from build123d import *

# Parameters (mm, degrees)
BASE_PLATE_SKETCH_W          = 140
BASE_PLATE_SKETCH_H          = 85
BASE_PLATE_DEPTH             = 18
UNDERSIDE_GROOVE_SKETCH_W    = 49
UNDERSIDE_GROOVE_SKETCH_H    = 3
UNDERSIDE_GROOVE_DEPTH       = 148.411838059
BASE_HOLES_SKETCH_R          = 8
BASE_HOLES_DEPTH             = 84.846586096
UPRIGHT_LUG_PLATE_DEPTH      = 12
UPRIGHT_LUG_PLATE_DEPTH_BACK = 24
UPRIGHT_LUG_PLATE_SKETCH_R   = 27.5
UPRIGHT_LUG_PLATE_SKETCH_R_2 = 15
SIDE_GUSSET_SKETCH_R         = 20
SIDE_GUSSET_SKETCH_R_2       = 9
SIDE_GUSSET_DEPTH            = 24
HINGE_BOSS_EXTENSION_DEPTH   = 12


with BuildPart() as part:
    # Base Plate Sketch → Base Plate (new body)
    with BuildSketch(Plane(origin=(0, 0, 0), x_dir=(1, 0, 0), z_dir=(0, 1, 0))):
        Rectangle(BASE_PLATE_SKETCH_W, BASE_PLATE_SKETCH_H)
    extrude(amount=BASE_PLATE_DEPTH)

    # Underside Groove Sketch → Underside Groove (cut, through all)
    with BuildSketch(Plane(origin=(70, 0, 0), x_dir=(0, 0, -1), z_dir=(1, 0, 0))):
        with Locations((0, 1.5)):
            Rectangle(UNDERSIDE_GROOVE_SKETCH_W, UNDERSIDE_GROOVE_SKETCH_H)
    extrude(amount=-UNDERSIDE_GROOVE_DEPTH, mode=Mode.SUBTRACT)

    # Base Holes Sketch → Base Holes (cut, through all)
    with BuildSketch(Plane(origin=(0, 18, 0), x_dir=(1, 0, 0), z_dir=(0, 1, 0))):
        with Locations(Location((-35, -12.5, 0), (0, 0, 270))):
            Circle(BASE_HOLES_SKETCH_R)
        with Locations(Location((35, -12.5, 0), (0, 0, 270))):
            Circle(BASE_HOLES_SKETCH_R)
    extrude(amount=-BASE_HOLES_DEPTH, mode=Mode.SUBTRACT)



with BuildPart() as body_2:
    # Upright Lug Plate Sketch → Upright Lug Plate (new, two sides: drawn at the far end of the back side and taken through both)
    with BuildSketch(Plane(origin=(0, 0, -42.5), x_dir=(-1, 0, 0), z_dir=(0, 0, -1)).offset(-UPRIGHT_LUG_PLATE_DEPTH_BACK)):
        with Locations((-20, 118)):
            Circle(UPRIGHT_LUG_PLATE_SKETCH_R)
        with Locations((-20, 118)):
            Circle(UPRIGHT_LUG_PLATE_SKETCH_R_2, mode=Mode.SUBTRACT)
    extrude(amount=UPRIGHT_LUG_PLATE_DEPTH + UPRIGHT_LUG_PLATE_DEPTH_BACK)


with BuildPart() as body_3:
    # Side Gusset Sketch → Side Gusset (new body)
    with BuildSketch(Plane(origin=(0, 0, -42.5), x_dir=(-1, 0, 0), z_dir=(0, 0, -1))):
        with Locations((50, 56)):
            Circle(SIDE_GUSSET_SKETCH_R)
        with Locations((50, 56)):
            Circle(SIDE_GUSSET_SKETCH_R_2, mode=Mode.SUBTRACT)
    extrude(amount=-SIDE_GUSSET_DEPTH)


with BuildPart() as part_1:
    add(part.part)

    add(body_2.part)  # Hinge Boss Extension merges body 2

    add(body_3.part)  # Hinge Boss Extension merges body 3
    # Hinge Boss Extension Sketch → Hinge Boss Extension (add)
    with BuildSketch(Plane(origin=(0, 0, -42.5), x_dir=(-1, 0, 0), z_dir=(0, 0, -1))):
        with BuildLine():
            Line((70, 18), (70, 56))
            ThreePointArc((70, 56), (40.100426872, 38.621897345), (39.800154813, 73.203579806))
            ThreePointArc((39.800154813, 73.203579806), (10.05246179, 76.375791932), (4.645420553, 105.799457153))
            ThreePointArc((4.645420553, 105.799457153), (-29.103509689, 92.050508457), (-46.866088482, 123.870544241))
            Line((-46.866088482, 123.870544241), (-70, 18))
            Line((-70, 18), (70, 18))
        make_face()
    extrude(amount=-HINGE_BOSS_EXTENSION_DEPTH)


solid = part_1.part
Input: part model. Units: mm. Frame: model coordinates. A direction names the side the tool comes from. Coordinates: 2 decimals unless noted, no trailing zeros. Write each loop counter-clockwise with the first axis right and the second up, starting at its lowest first coordinate (ties: lowest second). Pieces come first, ordered by that corner, then holes. Notation, with made-up numbers: M 29,-7 L 67,-7 A17 cw 67,6 Z; hole C 58,13 d10. An arc over 180 degrees is marked long. Answer as a JSON object with one key per item and string values. Group by question number.
(1) Section A-A on z = -28. Output: boundary loops of the cut face in (x, y), plus the area to 3 significant figures.
(2) Set-up query: faces 4 (the face through (-60.752, 72.864, -28.001)), 5 (the face through (-54, 47, -18.5)), 6 (the face through (-1, 0, 33)). Return all of +Z, -Z, +X, -X, +Y, -Y with unobstructed straight access to the full face (end or side cutting, diameter ignored); none if empty.
(3) Mould query, pull axis X, two halves, no side actions, for faces 1 (the face through (-1, 18, 5)), 2 (the face through (-10.384, 76.073, -36.584)), 3 (the face through (5.22, 141.19, -36.25)). Classes: pulls with the +X half, pulls with the -X half, needs draft (parallel to the pull), parting line crosses it, or undercut.
(4) Contact query for flat-ended pins moving along their axis: P1, Ø6, axis at x = 17, z = -35, coming from the +Y side; P2, Ø1, axis at x = -39, y = 52, coming from the -Z side; P3, Ø6, axis at y = 21.5, z = -39.5, coming from the +X side. Output: stop coordinate, or through.
(5) Ray query, line 1 along X through (y, z) = (8, 12); line 2 along Y through (x, z) = (20, -30); line 3 along Y through (x, z) = (20, -47). Return the intervals inside material, ascending. Write a range as [from, to].
(6) Section C-C on y = 59. Output: boundary loops of the cut face in (x, z), plus the area to 3 significant figures.
(7) Section D-D on x = -35. Output: boundary loops of the cut face in (y, z), plus the area to 3 significant figures.
(8) Section B-B on z = 12.5. Output: boundary loops of the cut face in (x, y).
Result set:
{
 "1": {"outline": "M -70,0 L 70,0 L 70,18 L -70,18 Z; C -50,56 d40; C 20,118 d55; hole C -50,56 d18; hole C 20,118 d30", "area": "5,190 mm2"},
 "2": {"face 4": "+Z", "face 5": "+Z, +X, -X, +Y", "face 6": "+Z, -Z, +X, -X, -Y"},
 "3": {"face 1": "needs draft", "face 2": "undercut", "face 3": "parting line crosses it"},
 "4": {"P1": "stops at y = 145.5", "P2": "stops at z = -42.5", "P3": "stops at x = 69.89"},
 "5": {"line 1": "x = [-70, -42.98], [-27.02, 27.02], [42.98, 70]", "line 2": "y = [0, 18], [90.5, 103], [133, 145.5]", "line 3": "y = [90.5, 103], [133, 145.5]"},
 "6": {"outline": "M -69.77,-42.5 L -58.49,-42.5 L -58.49,-18.5 L -69.77,-18.5 Z; M -41.51,-42.5 L 61.04,-42.5 L 61.04,-30.5 L -30.23,-30.5 L -30.23,-18.5 L -41.51,-18.5 Z", "area": "1,640 mm2"},
 "7": {"outline": "M 0,-42.5 L 71.01,-42.5 L 71.01,-30.5 L 69.23,-30.5 L 69.23,-18.5 L 42.77,-18.5 L 42.77,-30.5 L 18,-30.5 L 18,4.5 L 3,4.5 L 3,-24.5 L 0,-24.5 Z; M 0,24.5 L 3,24.5 L 3,20.5 L 18,20.5 L 18,42.5 L 0,42.5 Z", "area": "2,100 mm2"},
 "8": {"outline": "M -70,3 L -43,3 L -43,18 L -70,18 Z; M -27,3 L 27,3 L 27,18 L -27,18 Z; M 43,3 L 70,3 L 70,18 L 43,18 Z"}
}
